Source: three-view drawing plus pictorial views. Frame: mm from the lowest corner of the part. Round coordinates to 2 decimals unless told otherwise and drop trailing zeros. Order: outer loops, then holes, each group sorted by start corner. A loop starts at its lowest first (then second) coordinate and runs counter-clockwise, first axis right, second up. Notation, with made-up numbers: (46, 82) -> (62, 82) arc R15 ccw to (62, 107) -> close; hole circle Ø8 at (-7, 37.5). An arc over 180 degrees is marked (long way). Use a Markdown table: item, result.
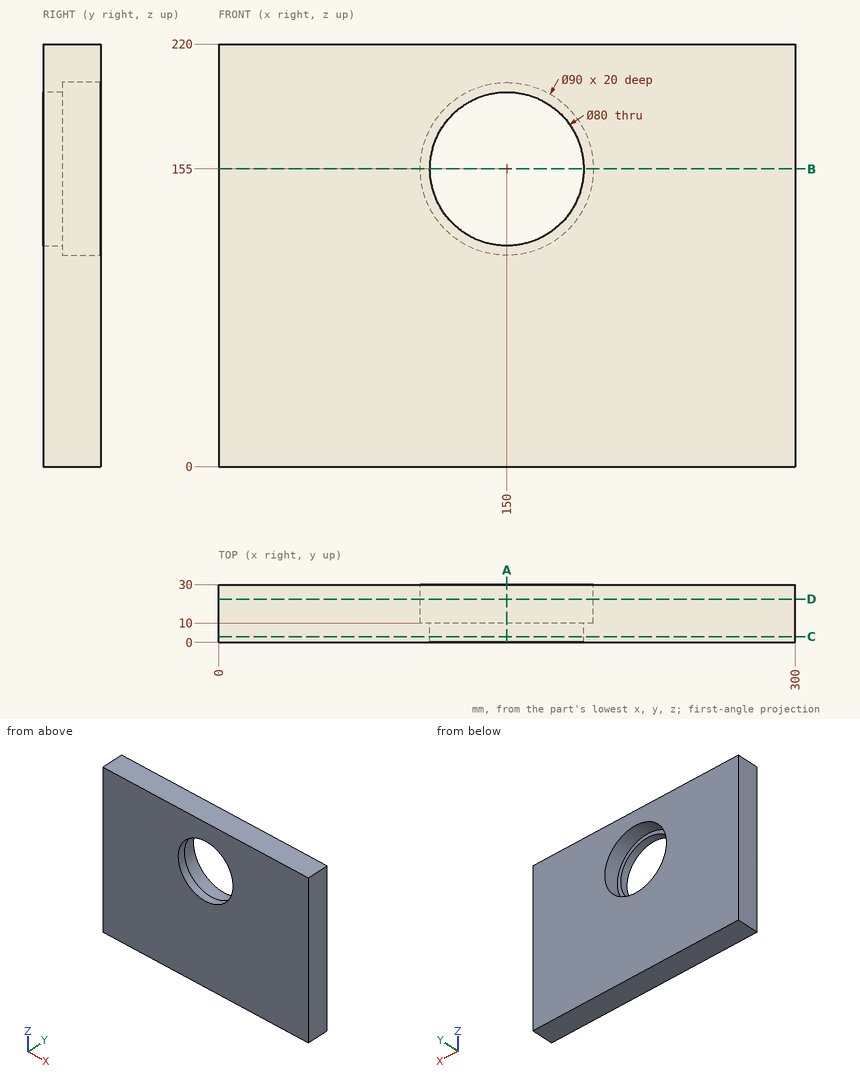
1) Cut plane A-A on x = 150. Return loops of the section in (y, z).
Results found:
| item | result |
|---|---|
| outline | (0, 0) -> (30, 0) -> (30, 110) -> (10, 110) -> (10, 115) -> (0, 115) -> close; (0, 195) -> (10, 195) -> (10, 200) -> (30, 200) -> (30, 220) -> (0, 220) -> close |
2) Cut plane B-B on z = 155. Return loops of the section in (x, y), and give its area (3 significant figures).
Results found:
| item | result |
|---|---|
| outline | (0, 0) -> (110, 0) -> (110, 10) -> (105, 10) -> (105, 30) -> (0, 30) -> close; (190, 0) -> (300, 0) -> (300, 30) -> (195, 30) -> (195, 10) -> (190, 10) -> close |
| area | 6,400 mm² |
3) Line query: L1, parallel to X at y = 4.5, z = 155; L2, parallel to X at y = 25.25, z = 155; L3, parallel to Z at x = 110.5, y = 13.5. Output: solid intervals per line, ascending. Write a range as [from, to].
Results found:
| item | result |
|---|---|
| L1 | x = [0, 110], [190, 300] |
| L2 | x = [0, 105], [195, 300] |
| L3 | z = [0, 133.44], [176.56, 220] |
4) Pin query (flat end, axial travel): pin 1 Ø5 at (y, z) = (12.5, 170) entering from -X. Return the tip coordinate at first contact, or that it passes through.
Results found:
| item | result |
|---|---|
| pin 1 | stops at x = 0 |
5) Cut plane C-C on y = 3. Return loops of the section in (x, z), and give its area (3 significant figures).
Results found:
| item | result |
|---|---|
| outline | (0, 0) -> (300, 0) -> (300, 220) -> (0, 220) -> close; hole circle Ø80 at (150, 155) |
| area | 61,000 mm² |
6) Cut plane D-D on y = 22.5. Return loops of the section in (x, z).
Results found:
| item | result |
|---|---|
| outline | (0, 0) -> (300, 0) -> (300, 220) -> (0, 220) -> close; hole circle Ø90 at (150, 155) |
